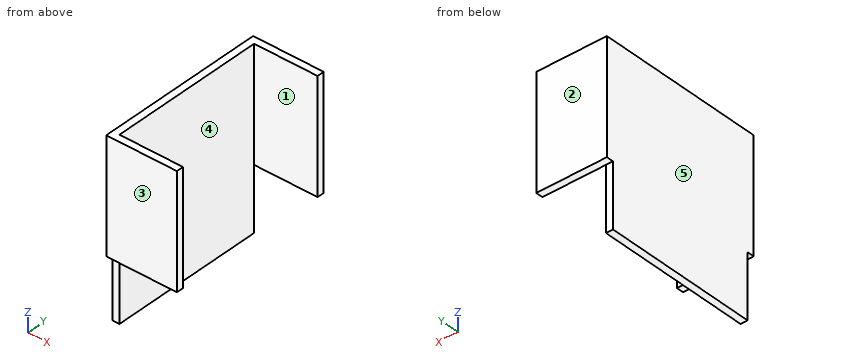
```python
from build123d import *

# Parameters (mm, degrees)
EXTRUDE_1_DEPTH     = 150
SKETCH_2_W          = 50
SKETCH_2_H          = 5
CUT_EXTRUDE_1_DEPTH = 45
SKETCH_3_W          = 5
SKETCH_3_H          = 110
CUT_EXTRUDE_2_DEPTH = 25
CUT_EXTRUDE_3_DEPTH = 25
CUT_EXTRUDE_4_DEPTH = 25


with BuildPart() as part:
    # 草图1 → 凸台-拉伸1 (new body)
    with BuildSketch(Plane.XY):
        Polygon((0, 0), (0, 120), (50, 120), (50, 115), (5, 115), (5, 5), (50, 5), (50, 0), align=None)
    extrude(amount=-EXTRUDE_1_DEPTH)

    # 草图2 → 切除-拉伸1 (cut)
    with BuildSketch(Plane(origin=(0, 0, -150), x_dir=(-1, 0, 0), z_dir=(0, 0, -1))):
        with Locations((-25, 117.5)):
            Rectangle(SKETCH_2_W, SKETCH_2_H)
        with Locations((-25, 2.5)):
            Rectangle(SKETCH_2_W, SKETCH_2_H)
    extrude(amount=-CUT_EXTRUDE_1_DEPTH, mode=Mode.SUBTRACT)

    # 草图3 → 切除-拉伸2 (cut)
    with BuildSketch(Plane(origin=(0, 0, -150), x_dir=(-1, 0, 0), z_dir=(0, 0, -1))):
        with Locations((-2.5, 60)):
            Rectangle(SKETCH_3_W, SKETCH_3_H)
    extrude(amount=-CUT_EXTRUDE_2_DEPTH, mode=Mode.SUBTRACT)

    # 草图4 → 切除-拉伸3 (cut)
    with BuildSketch(Plane(origin=(0, 0, -105), x_dir=(-1, 0, 0), z_dir=(0, 0, -1))):
        Polygon((-50, 120), (-50, 115), (-5, 115), (0, 115), (0, 120), align=None)
    extrude(amount=-CUT_EXTRUDE_3_DEPTH, mode=Mode.SUBTRACT)

    # 草图5 → 切除-拉伸4 (cut)
    with BuildSketch(Plane(origin=(0, 0, -105), x_dir=(-1, 0, 0), z_dir=(0, 0, -1))):
        Polygon((-50, 5), (-50, 0), (0, 0), (0, 5), (-5, 5), align=None)
    extrude(amount=-CUT_EXTRUDE_4_DEPTH, mode=Mode.SUBTRACT)


solid = part.part
```
Geometry: final body of the model. Coordinates: model frame, mm. Face numbers are marked on the shaded views. A direction names the side the tool comes from. Coordinates: 2 decimals unless noted, no trailing zeros. Order: outer loops, then holes, each group sorted by start corner. A loop starts at its lowest first (then second) coordinate and runs counter-clockwise, first axis right, second up. Notation, with made-up numbers: (37, 53) - (94, 53) arc R17 cw to (94, 58) - close; hole circle Ø11 at (19.5, 66). An arc over 180 degrees is marked (long way). Write each question's results on one line, items separated by ' | '.
(1) Section query C-C, the plane y = 84.5. Return the cut outline in (x, z).
Values found:
outline: (0, -125) - (5, -125) - (5, 0) - (0, 0) - close
(2) Section query B-B, the plane z = -62. Return the cut outline in (x, y), plus the area to 3 significant figures.
Values found:
outline: (0, 0) - (50, 0) - (50, 5) - (5, 5) - (5, 115) - (50, 115) - (50, 120) - (0, 120) - close | area: 1,050 mm²
(3) Mould query, pull axis Y, two halves, no side actions, for the marked faces 1, 2 and 3. Classes: +Y half, -Y half, draft (parallel to the pull), parting line (faces both ways), or undercut.
Values found:
face 1: undercut | face 2: +Y half | face 3: -Y half
(4) Set-up query: the marked faces 4 and 5. Return all of +Z, -Z, +X, -X, +Y, -Y with unobstructed straight access to the full face (end or side cutting, diameter ignored); none if empty.
Values found:
face 4: +Z, -Z, +X | face 5: +Z, -Z, -X, +Y, -Y
(5) Line query: line 1 (Y direction, x = 13.5, z = -35); line 2 (Z direction, x = 20, y = 115.5); line 3 (X direction, y = 83, z = -40). Output: solid intervals per line, ascending. Write a range as [from, to].
Values found:
line 1: y = [0, 5], [115, 120] | line 2: z = [-80, 0] | line 3: x = [0, 5]
(6) First-contact query: pin 1 Ø1.5 at (x, z) = (2, -96) entering from +Y; pin 2 Ø3 at (y, z) = (34.5, -16) entering from +X; pin 3 Ø4 at (x, y) = (25.5, 117.5) entering from -Z. Flat tips, straight axial feed; report the tip coordinate or a pass-through.
Values found:
pin 1: stops at y = 115 | pin 2: stops at x = 5 | pin 3: stops at z = -80
(7) Section query A-A, the plane x = 8.5. Return the cut outline in (y, z), plus the area to 3 significant figures.
Values found:
outline: (0, -80) - (5, -80) - (5, 0) - (0, 0) - close; (115, -80) - (120, -80) - (120, 0) - (115, 0) - close | area: 800 mm²
(8) Section query D-D, the plane z = -83. Return the cut outline in (x, y), plus the area to 3 significant figures.
Values found:
outline: (0, 5) - (5, 5) - (5, 115) - (0, 115) - close | area: 550 mm²
